Can you work these out from the model? Positions are in its coordinate system, mm. A direction names the side the tool comes from. Round coordinates to 2 decimals unless told otherwise and drop trailing zeros. Loops run counter-clockwise (first coordinate to the right, second up) from the corner with the lowest first, then second, coordinate; pieces in that order, holes last. Notation, with made-up numbers: (11.25, -16) -> (68.25, -16) arc R32 ccw to (68.25, 23) -> close; hole circle Ø5 at (21.5, 12). An arc over 180 degrees is marked (long way). Answer as a JSON object with one key per item and string values.
```python
from build123d import *

# Parameters (mm, degrees)
SKETCH_1_W      = 50
SKETCH_1_H      = 60
EXTRUDE_1_DEPTH = 50
SKETCH_2_R      = 17.5
EXTRUDE_2_DEPTH = 23
M30X2_0_1_D     = 28
M30X2_0_1_DEPTH = 20
M30X2_0_1_TIP   = 8.412048666
CHAMFER_1_SIZE  = 1


with BuildPart() as part:
    # 草图1 → 凸台-拉伸1 (new body)
    with BuildSketch(Plane.XY):
        Rectangle(SKETCH_1_W, SKETCH_1_H)
    extrude(amount=EXTRUDE_1_DEPTH)

    # 草图2 → 凸台-拉伸2 (add)
    with BuildSketch(Plane.XY.offset(50)):
        with Locations((0, -4.5)):
            Circle(SKETCH_2_R)
    extrude(amount=EXTRUDE_2_DEPTH)

    # M30x2.0 螺纹孔1
    with Locations(Plane(origin=(0, -30, 0), x_dir=(-1, 0, 0), z_dir=(0, -1, 0))):
        with Locations((0, -25)):
            Hole(M30X2_0_1_D / 2, depth=M30X2_0_1_DEPTH)
            with Locations((0, 0, -(M30X2_0_1_DEPTH + M30X2_0_1_TIP / 2))):  # 118° drill point
                Cone(0, M30X2_0_1_D / 2, M30X2_0_1_TIP, mode=Mode.SUBTRACT)

    # 倒角1
    chamfer_1_edges = [part.edges().sort_by_distance(p)[0] for p in [
        (-17.5, -4.5, 73),
    ]]
    chamfer(chamfer_1_edges, length=CHAMFER_1_SIZE)


solid = part.part
```
Q1. We'd pull the mould along Z, two halves only. Please class faces 1 (the conical face through (-2.25, -3.05, 25.93)), 2 (the flat face through (0, -4, 73)), 3 (the flat face through (-11, -30, 36)): pulls with the +Z half, pulls with the -Z half, needs draft (parallel to the pull), parting line crosses it, or undercut.
Determined:
{"face 1": "undercut", "face 2": "pulls with the +Z half", "face 3": "needs draft"}
Q2. I want a section at D-D, the plane y = 23. Write out the boundary of the cut face in (x, z), then the cut area to 3 significant figures.
Determined:
{"outline": "(-25, 0) -> (25, 0) -> (25, 50) -> (-25, 50) -> close", "area": "2,500 mm²"}
Q3. I want a section at B-B, the plane z = 54. Write out the boundary of the cut face in (x, y).
Determined:
{"outline": "circle Ø35 at (0, -4.5)"}
Q4. I want a section at C-C, the plane x = -22. Write out the boundary of the cut face in (y, z).
Determined:
{"outline": "(-30, 0) -> (30, 0) -> (30, 50) -> (-30, 50) -> close"}
Q5. If I drill on L1, parallel to Z at x = 0, y = -19; L2, parallel to Z at x = -13.5, y = 20.5; L3, parallel to X at y = -21.5, z = 23.5, over which ranges is the centre line in solid material (lowest first)? Write a range as [from, to].
Determined:
{"L1": "[0, 11], [39, 73]", "L2": "[0, 50]", "L3": "[-25, -13.92], [13.92, 25]"}
Q6. I'm going to push flat-ended pins straight in: pin 1 (3 mm diameter, centred on y = -5, z = 58, fed in from +X); pin 2 (3 mm diameter, centred on x = -16, y = 21, fed in from +Z). Where does each tip first touch, or does it pass through?
Determined:
{"pin 1": "x = 17.5", "pin 2": "z = 50"}
Q7. I want a section at A-A, the plane y = -4.5. Write out the boundary of the cut face in (x, z).
Determined:
{"outline": "(-25, 0) -> (25, 0) -> (25, 50) -> (17.5, 50) -> (17.5, 72) -> (16.5, 73) -> (-16.5, 73) -> (-17.5, 72) -> (-17.5, 50) -> (-25, 50) -> close; hole circle Ø9.69 at (0, 25)"}
Q8. On a 3-axis mill with a long thin cutter (end or side, diameter ignored), from which of +Z, -Z, +X, -X, +Y, -Y can I reach the whole of each face in a straight line? I mean faces 4 (the cylindrical face through (-3.03, -19.86, 38.67)), 5 (the cylindrical face through (-14, -15, 61)), 6 (the flat face through (0, 0, 0)). Say none if no direction works.
Determined:
{"face 4": "-Y", "face 5": "+Z", "face 6": "-Z, +X, -X, +Y, -Y"}
